For this review, take the finished solid that the model builds, in its own axes (mm). A direction names the side the tool comes from. Round coordinates to 2 decimals unless told otherwise and drop trailing zeros. Order: outer loops, then holes, each group sorted by start corner. A loop starts at its lowest first (then second) coordinate and runs counter-clockwise, first axis right, second up. Notation, with made-up numbers: M 5,-6 L 52,-6 A37 cw 52,32 Z; hole C 41.25,52.5 d9. An arc over 180 degrees is marked long. Answer in a Markdown table with one row per item. Add a question column.
```python
from build123d import *

# Parameters (mm, degrees)
BASE_PLATE_SKETCH_R      = 5.05
BASE_PLATE_DEPTH         = 2.7
LUG_SKETCH_W             = 5
LUG_SKETCH_H             = 12.3
LUG_DEPTH                = 20
LUG_WEB_DEPTH            = 5
FILLET_R2_3_R            = 2.3
PIN_HOLE_SKETCH_R        = 2.965
PIN_HOLE_5_93_DEPTH      = 5
COUNTERBORE_SKETCH_R     = 5
COUNTERBORE_10X2_5_DEPTH = 2.5


with BuildPart() as part:
    # Base Plate Sketch → Base Plate (new body)
    with BuildSketch(Plane(origin=(0, 0, 0), x_dir=(1, 0, 0), z_dir=(0, 1, 0))):
        with BuildLine():
            Line((-19.85, 10), (19.85, 10))
            ThreePointArc((19.85, 10), (29.85, 0), (19.85, -10))
            Line((19.85, -10), (-19.85, -10))
            ThreePointArc((-19.85, -10), (-29.85, 0), (-19.85, 10))
        make_face()
        with Locations(Location((-19.85, 0, 0), (0, 0, 90))):
            Circle(BASE_PLATE_SKETCH_R, mode=Mode.SUBTRACT)
        with Locations(Location((19.85, 0, 0), (0, 0, 90))):
            Circle(BASE_PLATE_SKETCH_R, mode=Mode.SUBTRACT)
    extrude(amount=BASE_PLATE_DEPTH)

    # Lug Sketch → Lug (add)
    with BuildSketch(Plane.XY.offset(10)):
        with Locations((-9.095, 8.85)):
            Rectangle(LUG_SKETCH_W, LUG_SKETCH_H)
    extrude(amount=-LUG_DEPTH)

    # Lug Web Sketch → Lug Web (add)
    with BuildSketch(Plane.ZY.offset(11.595)):
        with BuildLine():
            Line((-10, 15), (10, 15))
            ThreePointArc((10, 15), (0, 25), (-10, 15))
        make_face()
    extrude(amount=-LUG_WEB_DEPTH)

    # Base Plate Mirror: part across plane


with BuildPart() as part_1:
    add(part.part)
    add(part.part.mirror(Plane(origin=(0, 0, 0), x_dir=(0, 0, 1), z_dir=(1, 0, 0))))

    # Fillet R2.3
    fillet_r2_3_edges = [part_1.edges().sort_by_distance(p)[0] for p in [
        (-11.595, 2.7, 0),
        (11.595, 2.7, 0),
    ]]
    fillet(fillet_r2_3_edges, radius=FILLET_R2_3_R)

    # Pin Hole Sketch → Pin Hole Ø5.93 (cut)
    with BuildSketch(Plane.ZY.offset(11.595)):
        with Locations(Location((0, 15, 0), (0, 0, 270))):
            Circle(PIN_HOLE_SKETCH_R)
    pin_hole_5_93 = extrude(amount=-PIN_HOLE_5_93_DEPTH, mode=Mode.SUBTRACT)

    # Counterbore Sketch → Counterbore Ø10x2.5 (cut)
    with BuildSketch(Plane.ZY.offset(11.595)):
        with Locations(Location((0, 15, 0), (0, 0, 270))):
            Circle(COUNTERBORE_SKETCH_R)
    counterbore_10x2_5 = extrude(amount=-COUNTERBORE_10X2_5_DEPTH, mode=Mode.SUBTRACT)

    # Pin Hole Mirror: Pin Hole Ø5.93, Counterbore Ø10x2.5 across plane
    add(pin_hole_5_93.mirror(Plane(origin=(0, 0, 0), x_dir=(0, 0, 1), z_dir=(1, 0, 0))), mode=Mode.SUBTRACT)
    add(counterbore_10x2_5.mirror(Plane(origin=(0, 0, 0), x_dir=(0, 0, 1), z_dir=(1, 0, 0))), mode=Mode.SUBTRACT)


solid = part_1.part
```
1. The part is to be moulded in two halves that separate along Y. For faces 5 (the cylindrical face through (-10, 20, 0)), 6 (the cylindrical face through (-9, 25, 0)), 7 (the flat face through (0, 0, 0)), 8 (the cylindrical face through (10, 20, 0)), say which applies: pulls with the +Y half, pulls with the -Y half, needs draft (parallel to the pull), parting line crosses it, or undercut.
2. For faces 1 (the flat face through (6.595, 11.5, -0.1)), 2 (the flat face through (-9.095, 15.1, -3.3)), 3 (the flat face through (11.595, 13, -5)), 4 (the flat face through (-11.595, 13, -5)), list the 3-axis set-ups (+Z, -Z, +X, -X, +Y, -Y) from which the entire face can be reached by the end or side of a thin tool; tool diameter is ignored.
3. To check wall thickness, follow probe 1 along X at (y, z) = (10, -1.5) (3 decimals); probe 2 along Z at (x, y) = (19.85, 1.1); probe 3 along Z at (x, y) = (8, 15) (3 decimals). State the ranges of each line that lie inside material, in increasing order. Write a range as [from, to].
4. Consider section B-B on y = 4.25. Write out the cut boundary in (x, z) (3 decimals).
5. Consider section A-A on x = 21.5. Write out the cut boundary in (y, z).
6. Clearance check with flat-ended pins moving along their axes: pin 1 Ø8 at (y, z) = (16.5, -1.5) entering from -X (3 decimals); pin 2 Ø12 at (y, z) = (10.5, -5.5) entering from -X; pin 3 Ø6 at (y, z) = (15, 0) entering from -X (3 decimals); pin 4 Ø4.5 at (y, z) = (15, 0) entering from -X. State where each tip first meets the part, or that it passes through.
7. Consider section C-C on z = 0. State how many separate pieces and enclosed holes the cut face has, plus the area to 3 significant figures.
8. Consider section D-D on z = -6.5. Write out the cut boundary in (x, y) (3 decimals), plus the area to 3 significant figures.
Solved:
| question | item | result |
|---|---|---|
| 1 | face 5 | undercut |
| 1 | face 6 | pulls with the +Y half |
| 1 | face 7 | pulls with the -Y half |
| 1 | face 8 | undercut |
| 2 | face 1 | +Z, -Z, +Y |
| 2 | face 2 | -X |
| 2 | face 3 | +Z, -Z, +X, +Y |
| 2 | face 4 | +Z, -Z, -X, +Y |
| 3 | probe 1 | x = [-11.595, -6.595], [6.595, 11.595] |
| 3 | probe 2 | z = [-10, -5.05], [5.05, 10] |
| 3 | probe 3 | z = [-10, -2.965], [2.965, 10] |
| 4 | outline | M -11.721,-10 L -6.595,-10 L -6.595,10 L -11.721,10 Z; M 6.595,-10 L 11.721,-10 L 11.721,10 L 6.595,10 Z |
| 5 | outline | M 0,-9.86 L 2.7,-9.86 L 2.7,-4.77 L 0,-4.77 Z; M 0,4.77 L 2.7,4.77 L 2.7,9.86 L 0,9.86 Z |
| 6 | pin 1 | stops at x = -11.595 |
| 6 | pin 2 | stops at x = -11.65 |
| 6 | pin 3 | stops at x = -9.095 |
| 6 | pin 4 | passes through |
| 7 | separate pieces | 5 |
| 7 | enclosed holes | 0 |
| 7 | area | 252 mm^2 |
| 8 | outline | M -27.449,0 L 27.449,0 L 27.449,2.7 L 13.895,2.7 A2.3 cw 11.595,5 L 11.595,22.599 L 6.595,22.599 L 6.595,2.7 L -6.595,2.7 L -6.595,22.599 L -11.595,22.599 L -11.595,5 A2.3 cw -13.895,2.7 L -27.449,2.7 Z |
| 8 | area | 349 mm^2 |
